from build123d import *

# Parameters (mm, degrees)
SKETCH_2_R          = 1.25
CUT_EXTRUDE_1_DEPTH = 10


with BuildPart() as part:
    # 草图1 → 旋转1 (revolve)
    with BuildSketch(Plane.XY, mode=Mode.PRIVATE) as revolve_1_sk:
        Polygon((4, 4.368271468), (5, 4.368271468), (5, 3.368271468), (7, 3.368271468), (7, -1.631728532), (4, -1.631728532), align=None)
    revolve(revolve_1_sk.sketch.rotate(Axis((0, 0, 0), (0, 1, 0)), 90), axis=Axis((0, 0, 0), (0, 1, 0)))

    # 草图2 → 切除-拉伸1 (cut)
    with BuildSketch(Plane.XY):
        with Locations(Location((0, 0.868271468, 0), (0, 0, 270.000000001))):
            Circle(SKETCH_2_R)
    extrude(amount=-CUT_EXTRUDE_1_DEPTH, mode=Mode.SUBTRACT)


solid = part.part
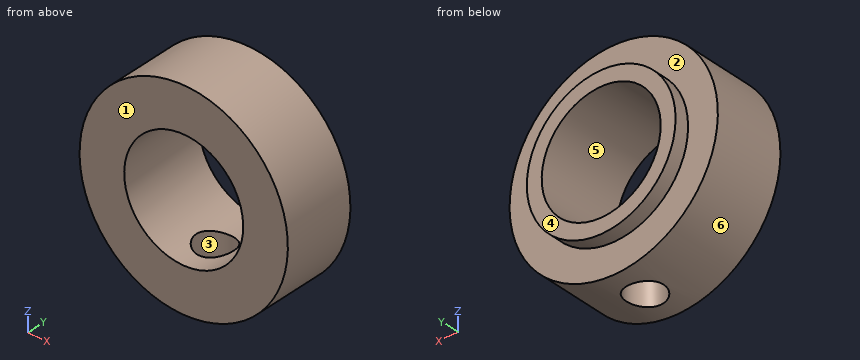
Could you check a few things on this model? Use its own coordinates, in mm. Face numbers are marked on the shaded views. A direction names the side the tool comes from. Give positions to 0.01 mm unless a question says otherwise; leave off trailing zeros. Loops run counter-clockwise (first coordinate to the right, second up) from the corner with the lowest first, then second, coordinate; pieces in that order, holes last. Notation, with made-up numbers: (-22, -38) -> (-4, -38) arc R26 ccw to (-4, -8) -> close; hole circle Ø10 at (11, 65.25). An arc over 180 degrees is marked (long way). Answer as CSV lines item,"result". Start each with the question number.
(1) We'd pull the mould along X, two halves only. Please class the marked faces 3, 4, 5 and 6: released by +X, released by -X, zero draft, split by the parting line, or undercut.
(2) Which directions (+Z, -Z, +X, -X, +Y, -Y) give clear straight access to the entire face, cutting with the end or side of a thin tool? Please do the marked faces 1 and 2.
(3) I need wall thicknesses on probe 1 along Y at (x, z) = (-2.25, 6); probe 2 along X at (y, z) = (2.25, -1); probe 3 along Z at (x, y) = (-2.25, 0.25). Which ranges of each line are inside material? Lowest first, please.
(4) If we section it at C-C on y = 4: Write out the boundary of the cut face in (x, z).
(5) If we section it at A-A on x = 0: Write out the boundary of the cut face in (y, z), then the cut area to 3 significant figures.
(6) I'm going to push flat-ended pins straight in: pin 1 Ø6.5 at (x, z) = (0, 0) entering from +Y; pin 2 Ø1 at (y, z) = (0, 3.5) entering from +X; pin 3 Ø1 at (y, z) = (2.5, -2.5) entering from +X; pin 4 Ø1 at (x, z) = (-4, -4) entering from +Y. Where does each tip first touch, or does it pass through?
(7) If we section it at B-B on z = 0: Write out the boundary of the cut face in (x, y).
(8) If we section it at D-D on x = 2.5: Write out the boundary of the cut face in (y, z).
Computed:
1,face 3,"undercut"
1,face 4,"zero draft"
1,face 5,"undercut"
1,face 6,"split by the parting line"
2,face 1,"+Z, -Z, +X, -X, -Y"
2,face 2,"+Y"
3,probe 1,"y = -1.63 to 3.37"
3,probe 2,"x = -6.93 to -3.87, 3.87 to 6.93"
3,probe 3,"z = -6.63 to -3.31, 3.31 to 6.63"
4,outline,"circle Ø10 at (0, 0); hole circle Ø8 at (0, 0)"
5,outline,"(-1.63, -7) -> (-0.38, -7) -> (-0.38, -4) -> (-1.63, -4) -> close; (-1.63, 4) -> (4.37, 4) -> (4.37, 5) -> (3.37, 5) -> (3.37, 7) -> (-1.63, 7) -> close; (2.12, -7) -> (3.37, -7) -> (3.37, -5) -> (4.37, -5) -> (4.37, -4) -> (2.12, -4) -> close"
5,area,"24.5 mm2"
6,pin 1,"passes through"
6,pin 2,"stops at x = 6.32"
6,pin 3,"stops at x = 6.71"
6,pin 4,"stops at y = 3.37"
7,outline,"(-7, -1.63) -> (-4, -1.63) -> (-4, 4.37) -> (-5, 4.37) -> (-5, 3.37) -> (-7, 3.37) -> close; (4, -1.63) -> (7, -1.63) -> (7, 3.37) -> (5, 3.37) -> (5, 4.37) -> (4, 4.37) -> close"
8,outline,"(-1.63, -6.54) -> (3.37, -6.54) -> (3.37, -4.33) -> (4.37, -4.33) -> (4.37, -3.12) -> (-1.63, -3.12) -> close; (-1.63, 3.12) -> (4.37, 3.12) -> (4.37, 4.33) -> (3.37, 4.33) -> (3.37, 6.54) -> (-1.63, 6.54) -> close"
